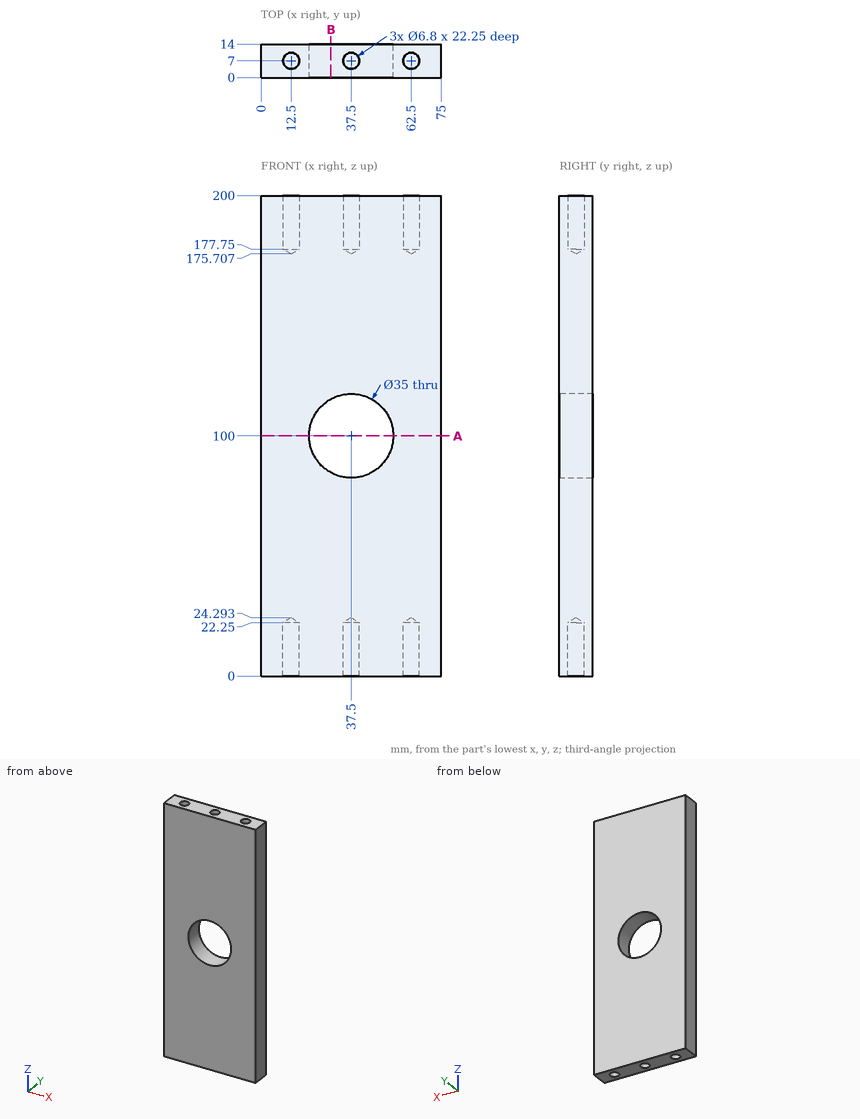
Answer from the drawing. Dimensions are ordinates in mm from the lowest x, y and z of the part. Coordinates: 2 decimals unless noted, no trailing zeros. Write each loop counter-clockwise with the first axis right and the second up, starting at its lowest first coordinate (ties: lowest second). Pieces come first, ordered by that corner, then holes. Notation, with made-up numbers: M 31.5,-21 L 85.5,-21 A13 cw 85.5,-10 Z; hole C -2,23 d2. An arc over 180 degrees is marked long. Write item = value, one per line.
1. The part is cut by section A-A (z = 100). Determine the outline of the cut face in (x, y), then the cut area to 3 significant figures.
Solution:
outline = M 0,0 L 20,0 L 20,14 L 0,14 Z; M 55,0 L 75,0 L 75,14 L 55,14 Z
area = 560 mm2
2. Flat-ended cylindrical pins translate along their axes: pin 1 (8 mm diameter, centred on x = 12.5, y = 7, fed in from +Z); pin 2 (4 mm diameter, centred on x = 62.5, y = 7, fed in from +Z); pin 3 (5.5 mm diameter, centred on x = 12.5, y = 7, fed in from -Z). Find the tip coordinate at first contact, or state that the pin passes through.
Solution:
pin_1 = 200
pin_2 = 176.91
pin_3 = 22.64
3. The part is cut by section B-B (x = 29). Determine the outline of the cut face in (y, z), then the cut area to 3 significant figures.
Solution:
outline = M 0,0 L 14,0 L 14,84.7 L 0,84.7 Z; M 0,115.3 L 14,115.3 L 14,200 L 0,200 Z
area = 2,370 mm2
4. Straight lines are drawn through the part: line 1 (X direction, y = 7, z = 17.5); line 2 (Y direction, x = 12, z = 14); line 3 (Z direction, x = 39, y = 11.5). For each, find the intervals that lie inside material, in ascending order. Write a range as from..to.
Solution:
line_1 = 0..9.1, 15.9..34.1, 40.9..59.1, 65.9..75
line_2 = 0..3.64, 10.36..14
line_3 = 0..82.56, 117.44..200
